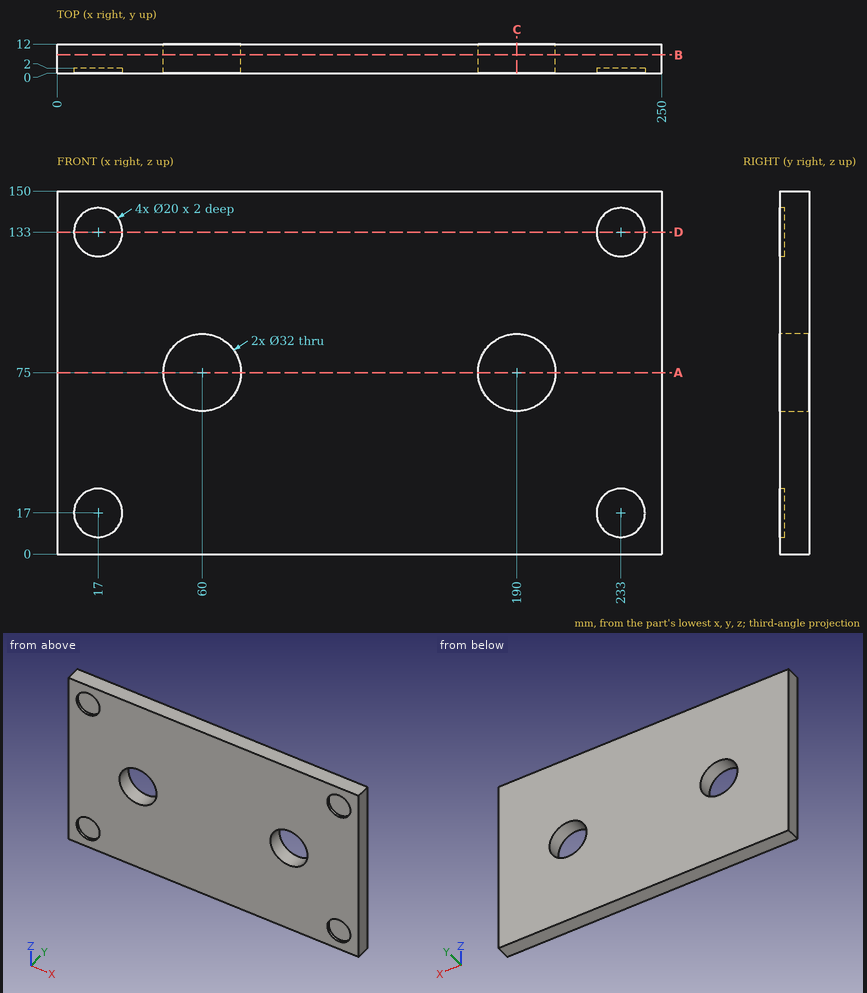
Could you check a few things on this drawing? It's one solid part, dimensions in mm from its lowest x, y, z. Round coordinates to 2 decimals unless told otherwise and drop trailing zeros. Loops run counter-clockwise (first coordinate to the right, second up) from the corner with the lowest first, then second, coordinate; pieces in that order, holes last. Notation, with made-up numbers: M -23.5,21.25 L -16.5,21.25 A20 cw -16.5,48.25 Z; hole C 21,9.5 d7. An arc over 180 degrees is marked long. Write item = value, one per line. Start each with the question number.
(1) I need wall thicknesses on line 1 along X through (y, z) = (6, 75); line 2 along X through (y, z) = (1.45, 17); line 3 along Z through (x, y) = (57, 10). Which ranges of each line are inside material? Lowest first, please.
(2) Suppose I cut it at A-A on z = 75. Write out the boundary of the cut face in (x, y).
(3) Suppose I cut it at D-D on z = 133. Write out the boundary of the cut face in (x, y), plus the area to 3 significant figures.
(4) I'm going to push a flat-ended pin straight in: P1, Ø6, axis at x = 237.5, z = 131, coming from the -Y side. Where does the tip first touch, or does it pass through?
(5) Suppose I cut it at C-C on x = 190. Write out the boundary of the cut face in (y, z), plus the area to 3 significant figures.
(6) Suppose I cut it at B-B on y = 7.5. Write out the boundary of the cut face in (x, z).
Answer block:
q1.line_1 = 0 to 44, 76 to 174, 206 to 250
q1.line_2 = 0 to 7, 27 to 223, 243 to 250
q1.line_3 = 0 to 59.28, 90.72 to 150
q2.outline = M 0,0 L 44,0 L 44,12 L 0,12 Z; M 76,0 L 174,0 L 174,12 L 76,12 Z; M 206,0 L 250,0 L 250,12 L 206,12 Z
q3.outline = M 0,0 L 7,0 L 7,2 L 27,2 L 27,0 L 223,0 L 223,2 L 243,2 L 243,0 L 250,0 L 250,12 L 0,12 Z
q3.area = 2,920 mm²
q4.P1 = 2
q5.outline = M 0,0 L 12,0 L 12,59 L 0,59 Z; M 0,91 L 12,91 L 12,150 L 0,150 Z
q5.area = 1,420 mm²
q6.outline = M 0,0 L 250,0 L 250,150 L 0,150 Z; hole C 60,75 d32; hole C 190,75 d32
